```python
from build123d import *

# Parameters (mm, degrees)
SKETCH_1_R      = 10
EXTRUDE_1_DEPTH = 5


with BuildPart() as part:
    # 草图1 → 凸台-拉伸1 (new, symmetric)
    with BuildSketch(Plane(origin=(0, 0, 0), x_dir=(1, 0, 0), z_dir=(0, 1, 0))):
        with BuildLine():
            Line((-20, -23.285), (20, -23.285))
            Line((20, -23.285), (20, 23.285))
            ThreePointArc((20, 23.285), (0, 43.285), (-20, 23.285))
            Line((-20, 23.285), (-20, -23.285))
        make_face()
        with Locations(Location((0, 23.285, 0), (0, 0, 270))):
            Circle(SKETCH_1_R, mode=Mode.SUBTRACT)
    extrude(amount=EXTRUDE_1_DEPTH, both=True)


solid = part.part
```
Part model, mm, in its own coordinate system. Round coordinates to 2 decimals unless told otherwise and drop trailing zeros. Write each loop counter-clockwise with the first axis right and the second up, starting at its lowest first coordinate (ties: lowest second). Pieces come first, ordered by that corner, then holes. Notation, with made-up numbers: (83, 27) -> (126, 27) arc R15 ccw to (126, 49) -> close; hole circle Ø5 at (22.25, -16.75). An arc over 180 degrees is marked (long way). Return JSON: item names as keys, results as strings. Group by question number.
Q1. Mould opens along Z. For faces 1 (the cylindrical face through (0.44, 0.07, -43.28)), 2 (the flat face through (0, 0, 23.285)), 3 (the flat face through (0, -5, -3)), 4 (the cylindrical face through (3.004, -0.07, -13.747)) say: pulls with the +Z half, pulls with the -Z half, needs draft (parallel to the pull), parting line crosses it, or undercut.
Q2. Saw through at C-C on y = -2.75. Write the cut outline in (x, z) (3 decimals), plus the area to 3 significant figures.
Q3. Saw through at D-D on x = 11. Write the cut outline in (y, z) (3 decimals).
Q4. Saw through at A-A on x = 0. Write the cut outline in (y, z) (3 decimals).
Q5. Probe L1, parallel to Z at x = 4.5, y = -1.5 (3 decimals); L2, parallel to Z at x = -8, y = 0.75 (3 decimals); L3, parallel to X at y = 3.25, z = -27. List the from-to ranges inside material, lowest first. Write a range as [from, to].
Q6. Saw through at B-B on z = -29. Write the cut outline in (x, y), plus the area to 3 significant figures.
Answer:
{
 "1": {"face 1": "pulls with the -Z half", "face 2": "pulls with the +Z half", "face 3": "needs draft", "face 4": "undercut"},
 "2": {"outline": "(-20, -23.285) arc R20 ccw to (20, -23.285) -> (20, 23.285) -> (-20, 23.285) -> close; hole circle Ø20 at (0, -23.285)", "area": "2,180 mm2"},
 "3": {"outline": "(-5, -39.988) -> (5, -39.988) -> (5, 23.285) -> (-5, 23.285) -> close"},
 "4": {"outline": "(-5, -43.285) -> (5, -43.285) -> (5, -33.285) -> (-5, -33.285) -> close; (-5, -13.285) -> (5, -13.285) -> (5, 23.285) -> (-5, 23.285) -> close"},
 "5": {"L1": "[-42.772, -32.215], [-14.355, 23.285]", "L2": "[-41.615, -29.285], [-17.285, 23.285]", "L3": "[-19.65, -9.28], [9.28, 19.65]"},
 "6": {"outline": "(-19.17, -5) -> (-8.21, -5) -> (-8.21, 5) -> (-19.17, 5) -> close; (8.21, -5) -> (19.17, -5) -> (19.17, 5) -> (8.21, 5) -> close", "area": "219 mm2"}
}
